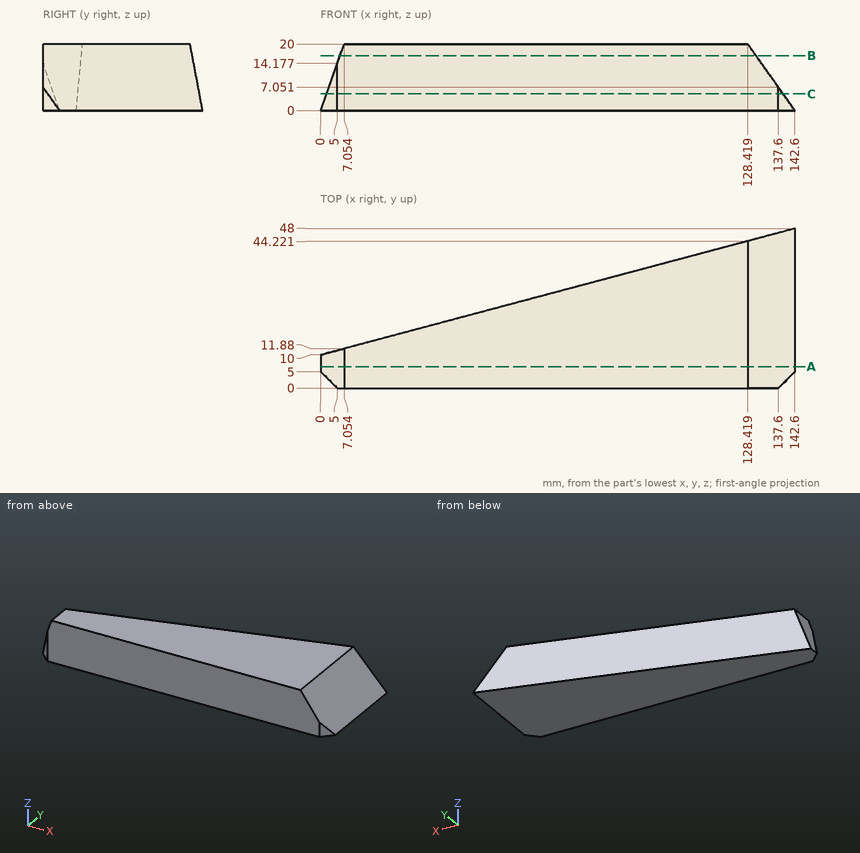
Verification items for this drawing (mm, ordinates from the low corner). Coordinates: 2 decimals unless noted, no trailing zeros. Order: outer loops, then holes, each group sorted by start corner. A loop starts at its lowest first (then second) coordinate and runs counter-clockwise, first axis right, second up. Notation, with made-up numbers: (-28, -40) - (4, -40) arc R19 ccw to (4, -6) - close; hole circle Ø5 at (32, 42). An arc over 180 degrees is marked (long way). Use one line per item in the form item = value.
1. Section check C-C (z = 5). Record the boundary of the cut face in (x, y) (1 decimal).
Here are the results:
outline = (1.8, 3.2) - (5, 0) - (137.6, 0) - (139.1, 1.5) - (139.1, 47.1) - (1.8, 10.5) - close
2. Section check B-B (z = 16.5). Record the boundary of the cut face in (x, y).
Here are the results:
outline = (5.82, 0) - (130.9, 0) - (130.9, 44.88) - (5.82, 11.55) - close
3. Gauge pin test, flat ends, axial feed: pin 1 (3 mm diameter, centred on y = 42.5, z = 10.5, fed in from +X); pin 2 (6 mm diameter, centred on x = 44, y = 27.5, fed in from -Z); pin 3 (8 mm diameter, centred on x = 50.5, z = 14, fed in from +Y). Record the tip position at first contact, or that the pin passes through.
Here are the results:
pin_1 = 136.22
pin_2 = through
pin_3 = 24.52
4. Section check A-A (y = 6.5). Record the boundary of the cut face in (x, z).
Here are the results:
outline = (0, 0) - (142.6, 0) - (128.42, 20) - (7.05, 20) - close
5. Scan lines: line 1 (Y direction, x = 58, z = 17) (1 decimal); line 2 (Y direction, x = 93, z = 12.5); line 3 (Z direction, x = 137, y = 28) (1 decimal). Record each from-to range of solid material in increasing order.
Here are the results:
line_1 = 0 to 25.5
line_2 = 0 to 34.78
line_3 = 0 to 7.9
